Source: CAD feature listing. Evaluate the final solid. Frame: model axes, mm. Round coordinates to 2 decimals unless told otherwise and drop trailing zeros. Order: outer loops, then holes, each group sorted by start corner. A loop starts at its lowest first (then second) coordinate and runs counter-clockwise, first axis right, second up. Notation, with made-up numbers: (-7.5, 57) - (23.5, 57) arc R16 cw to (23.5, 62) - close; hole circle Ø1 at (11.5, 75). An arc over 180 degrees is marked (long way). Return JSON: item names as keys, results as strings. Group by question number.
1) Section B-B, the plane z = 93.5. Return loops of the section in (x, y), plus the area to 3 significant figures.
2) Section C-C, the plane x = -340. Return loops of the section in (y, z).
3) Ray query, line 1 (X direction, y = 23.5, z = -470.5); line 2 (Z direction, x = 8, y = 20); line 3 (Z direction, x = -228, y = 14.5). Return the intervals inside material, ascending. Write a range as from..to.
4) Section A-A, the plane y = 16.5. Give the number of separate pieces and of enclosed holes in the cut face, plus the area to 3 significant figures.
5) Contact query for flat-ended pins moving along their axis: P1, Ø1, axis at x = 521.5, y = 20.5, coming from the +Z side; P2, Ø21, axis at x = -241.03, z = -741.82, coming from the +Y side; P3, Ø6, axis at y = 4, z = -598, coming from the +X side; P4, Ø3, axis at x = -153, y = 19.5, coming from the +Z side. Output: stop coordinate, or through.
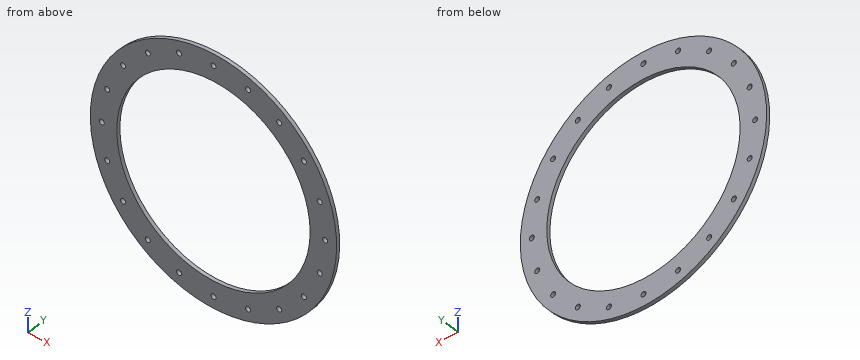
```python
from build123d import *

# Parameters (mm, degrees)
SKETCH_1_R                = 860
SKETCH_1_R_2              = 675
EXTRUDE_1_DEPTH           = 25
HOLE_WIZARD_25_5_25_5_1_D = 35


with BuildPart() as part:
    # 草图1 → 凸台-拉伸1 (new body)
    with BuildSketch(Plane(origin=(0, 0, 0), x_dir=(1, 0, 0), z_dir=(0, 1, 0))):
        with Locations(Location((0, 0, 0), (0, 0, 270))):
            Circle(SKETCH_1_R)
        with Locations(Location((0, 0, 0), (0, 0, 270))):
            Circle(SKETCH_1_R_2, mode=Mode.SUBTRACT)
    extrude(amount=EXTRUDE_1_DEPTH)

    # Ø25.5 (25.5) 直径孔1 (through all)
    with Locations(Plane(origin=(0, 25, 0), x_dir=(1, 0, 0), z_dir=(0, 1, 0))):
        with Locations((0, 780), (241.033255612, 741.82408271), (458.472496788, 631.033255612), (631.033255612, 458.472496788), (741.82408271, 241.033255612), (780, 0), (741.82408271, -241.033255612), (631.033255612, -458.472496788), (458.472496788, -631.033255612), (241.033255612, -741.82408271), (0, -780), (-241.033255612, -741.82408271), (-458.472496788, -631.033255612), (-631.033255612, -458.472496788), (-741.82408271, -241.033255612), (-780, 0), (-741.82408271, 241.033255612), (-631.033255612, 458.472496788), (-458.472496788, 631.033255612), (-241.033255612, 741.82408271)):
            Hole(HOLE_WIZARD_25_5_25_5_1_D / 2)


solid = part.part
```
Geometry check:
{
 "1": {"outline": "(-854.9, 0) - (-668.49, 0) - (-668.49, 25) - (-854.9, 25) - close; (668.49, 0) - (854.9, 0) - (854.9, 25) - (668.49, 25) - close", "area": "9,320 mm2"},
 "2": {"outline": "(0, -789.94) - (25, -789.94) - (25, -583.12) - (0, -583.12) - close; (0, 583.12) - (25, 583.12) - (25, 789.94) - (0, 789.94) - close"},
 "3": {"line 1": "-719.88..-643.75, -618.32..-484, 484..618.32, 643.75..719.88", "line 2": "-859.96..-795.56, -764.44..-674.95, 674.95..764.44, 795.56..859.96", "line 3": "-829.23..-753.5, -730.15..-635.33, 635.33..730.15, 753.5..829.23"},
 "4": {"separate pieces": "1", "enclosed holes": "21", "area": "873,000 mm2"},
 "5": {"P1": "z = 684.22", "P2": "through", "P3": "x = 620.95", "P4": "z = 846.55"}
}
